from build123d import *

# Parameters (mm, degrees)
SKETCH_1_W                   = 60
SKETCH_1_H                   = 30
EXTRUDE_1_DEPTH              = 90
M16X1_5_1_D                  = 14.5
HOLE_WIZARD_M6_1_D           = 6.6
HOLE_WIZARD_M6_1_CBORE_D     = 11
HOLE_WIZARD_M6_1_CBORE_DEPTH = 30
CHAMFER_1_SIZE               = 2


with BuildPart() as part:
    # 草图1 → 凸台-拉伸1 (new body)
    with BuildSketch(Plane.XY):
        Rectangle(SKETCH_1_W, SKETCH_1_H)
    extrude(amount=EXTRUDE_1_DEPTH)

    # M16x1.5 螺纹孔1 (through all)
    with Locations(Plane(origin=(0, -15, 0), x_dir=(-1, 0, 0), z_dir=(0, -1, 0))):
        with Locations((0, -19)):
            Hole(M16X1_5_1_D / 2)

    # M6 六角凹头螺钉的柱形沉头孔1 (through all)
    with Locations(Plane(origin=(0, 0, 0), x_dir=(-1, 0, 0), z_dir=(0, 0, -1))):
        with Locations((22, -7.5), (22, 7.5), (-22, 7.5), (-22, -7.5)):
            CounterBoreHole(HOLE_WIZARD_M6_1_D / 2, HOLE_WIZARD_M6_1_CBORE_D / 2, HOLE_WIZARD_M6_1_CBORE_DEPTH)

    # 倒角1
    chamfer_1_edges = [part.edges().sort_by_distance(p)[0] for p in [
        (30, -15, 45),
        (-30, -15, 45),
        (-30, 15, 45),
        (30, 15, 45),
    ]]
    chamfer(chamfer_1_edges, length=CHAMFER_1_SIZE)


solid = part.part
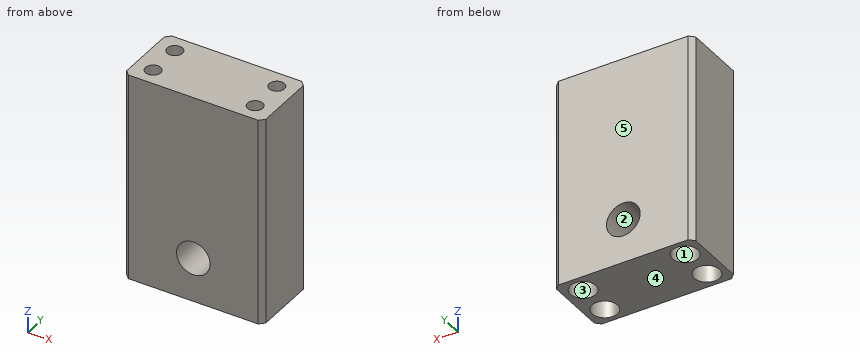
Could you check a few things on this model? Use its own coordinates, in mm. Face numbers are marked on the shaded views. A direction names the side the tool comes from. Give positions to 0.01 mm unless a question says otherwise; leave off trailing zeros. Order: outer loops, then holes, each group sorted by start corner. A loop starts at its lowest first (then second) coordinate and runs counter-clockwise, first axis right, second up.
1. I need wall thicknesses on L1, parallel to Y at x = 22, z = 65; L2, parallel to Y at x = -22, z = 24; L3, parallel to X at y = -9.25, z = 47. Which ranges of each line are inside material? Lowest first, please.
2. We'd pull the mould along Y, two halves only. Please class the marked faces 3, 4 and 5: pulls with the +Y half, pulls with the -Y half, needs draft (parallel to the pull), parting line crosses it, or undercut.
3. Suppose I cut it at C-C (z = 22.5). List the corners of the cut face in (x, y) for me.
4. Suppose I cut it at D-D (z = 71.5). List the corners of the cut face in (x, y) for me, plus the area to 3 significant figures.
5. Suppose I cut it at B-B (x = -22). List the corners of the cut face in (y, z) for me.
6. For the marked faces 1 and 2, which set-ups out of +Z, -Z, +X, -X, +Y, -Y let a thin tool reach every point of the face, with its end or its side?
7. Suppose I cut it at A-A (y = 7.5). List the corners of the cut face in (x, z) for me.
8. Will these pins go through, and if not, where does the flat tip stop? P1, Ø7.5, axis at x = 22, y = 7.5, coming from the -Z side; P2, Ø5.5, axis at x = -20, y = 5.5, coming from the -Z side.
Solved:
1. L1: y = -15 to -10.8, -4.2 to 4.2, 10.8 to 15
1. L2: y = -15 to -13, -2 to 2, 13 to 15
1. L3: x = -30 to -24.8, -19.2 to 19.2, 24.8 to 30
2. face 3: undercut
2. face 4: needs draft
2. face 5: pulls with the +Y half
3. outline: (-30, -13) - (-28, -15) - (-6.35, -15) - (-6.35, 15) - (-28, 15) - (-30, 13) - close; (6.35, -15) - (28, -15) - (30, -13) - (30, 13) - (28, 15) - (6.35, 15) - close; hole circle Ø11 at (-22, -7.5); hole circle Ø11 at (-22, 7.5); hole circle Ø11 at (22, -7.5); hole circle Ø11 at (22, 7.5)
4. outline: (-30, -13) - (-28, -15) - (28, -15) - (30, -13) - (30, 13) - (28, 15) - (-28, 15) - (-30, 13) - close; hole circle Ø6.6 at (-22, -7.5); hole circle Ø6.6 at (-22, 7.5); hole circle Ø6.6 at (22, -7.5); hole circle Ø6.6 at (22, 7.5)
4. area: 1,660 mm2
5. outline: (-15, 0) - (-13, 0) - (-13, 30) - (-10.8, 30) - (-10.8, 90) - (-15, 90) - close; (-4.2, 30) - (-2, 30) - (-2, 0) - (2, 0) - (2, 30) - (4.2, 30) - (4.2, 90) - (-4.2, 90) - close; (10.8, 30) - (13, 30) - (13, 0) - (15, 0) - (15, 90) - (10.8, 90) - close
6. face 1: -Z
6. face 2: +Y, -Y
7. outline: (-30, 0) - (-27.5, 0) - (-27.5, 30) - (-25.3, 30) - (-25.3, 90) - (-30, 90) - close; (-18.7, 30) - (-16.5, 30) - (-16.5, 0) - (16.5, 0) - (16.5, 30) - (18.7, 30) - (18.7, 90) - (-18.7, 90) - close; (25.3, 30) - (27.5, 30) - (27.5, 0) - (30, 0) - (30, 90) - (25.3, 90) - close; hole circle Ø14.5 at (0, 19)
8. P1: stops at z = 30
8. P2: stops at z = 0
